Input: part model. Units: mm. Frame: model coordinates. Coordinates: 2 decimals unless noted, no trailing zeros. Loops run counter-clockwise (first coordinate to the right, second up) from the corner with the lowest first, then second, coordinate; pieces in that order, holes last.
Item 1: Pull-direction query (Y, two-part tool) for faces 1 (the cylindrical face through (-66.616, 90.513, 0.028)), 2 (the flat face through (-3, -34, -2)), 3 (the cylindrical face through (-1.73, -7.81, 0.03)); classes: released by +Y, released by -Y, zero draft, split by the parting line, or undercut.
Item 2: Section A-A on x = 0. Return loops of the section in (y, z), and give its area (3 significant figures).
Item 3: Section B-B on y = 80. Return loops of the section in (x, z).
Item 4: Section C-C on z = 0.6. Return loops of the section in (x, y), and give its area (3 significant figures).
Item 5: Ray query, line 1 along Y through (x, z) = (0, -1.1); line 2 along Y through (x, z) = (-100, -0.7); line 3 along X through (y, z) = (0, -0.15). Return the intervals inside material, ascending.
Item 6: Contact query for a flat-ended pin moving along its axis: P1, Ø14.5, axis at x = 0, y = 0, coming from the +Z side. Output: stop coordinate, or through.
```python
from build123d import *

# Parameters (mm, degrees)
SKETCH_1_W          = 386
SKETCH_1_H          = 326
EXTRUDE_1_DEPTH     = 2
SKETCH_2_R          = 8
SKETCH_2_R_2        = 35
CUT_EXTRUDE_1_DEPTH = 12


with BuildPart() as part:
    # 草图1 → 凸台-拉伸1 (new, symmetric)
    with BuildSketch(Plane.XY):
        Rectangle(SKETCH_1_W, SKETCH_1_H)
    extrude(amount=EXTRUDE_1_DEPTH, both=True)

    # 草图2 → 切除-拉伸1 (cut, symmetric)
    with BuildSketch(Plane.XY):
        Circle(SKETCH_2_R)
        with Locations((-100, 80)):
            Circle(SKETCH_2_R_2)
    extrude(amount=CUT_EXTRUDE_1_DEPTH, both=True, mode=Mode.SUBTRACT)


solid = part.part
```
Results found:
1. face 1: undercut
1. face 2: zero draft
1. face 3: undercut
2. outline: (-163, -2) - (-8, -2) - (-8, 2) - (-163, 2) - close; (8, -2) - (163, -2) - (163, 2) - (8, 2) - close
2. area: 1,240 mm2
3. outline: (-193, -2) - (-135, -2) - (-135, 2) - (-193, 2) - close; (-65, -2) - (193, -2) - (193, 2) - (-65, 2) - close
4. outline: (-193, -163) - (193, -163) - (193, 163) - (-193, 163) - close; hole circle Ø70 at (-100, 80); hole circle Ø16 at (0, 0)
4. area: 122,000 mm2
5. line 1: y = -163 to -8, 8 to 163
5. line 2: y = -163 to 45, 115 to 163
5. line 3: x = -193 to -8, 8 to 193
6. P1: passes through
